Part model, mm, in its own coordinate system. Give positions to 0.01 mm unless a question says otherwise; leave off trailing zeros. Order: outer loops, then holes, each group sorted by start corner. A loop starts at its lowest first (then second) coordinate and runs counter-clockwise, first axis right, second up. Notation, with made-up numbers: (76.5, 14) - (93.5, 14) arc R15 ccw to (93.5, 20) - close; hole circle Ø2 at (39.5, 57.5). An arc over 180 degrees is marked (long way). Use a Markdown table: item, result. Add a question column.
from build123d import *

# Parameters (mm, degrees)
SKETCH_1_W         = 180
SKETCH_1_H         = 60
EXTRUDE_1_DEPTH    = 60
HOLE_WIZARD_M4_1_D = 4.8


with BuildPart() as part:
    # 草图1 → 凸台-拉伸1 (new body)
    with BuildSketch(Plane(origin=(0, 0, 0), x_dir=(1, 0, 0), z_dir=(0, 1, 0))):
        Rectangle(SKETCH_1_W, SKETCH_1_H)
    extrude(amount=EXTRUDE_1_DEPTH)

    # M4 间隙孔1 (through all)
    with Locations(Plane(origin=(0, 0, -30), x_dir=(-1, 0, 0), z_dir=(0, 0, -1))):
        with Locations((0, 30), (50, 30), (-50, 30)):
            Hole(HOLE_WIZARD_M4_1_D / 2)


solid = part.part
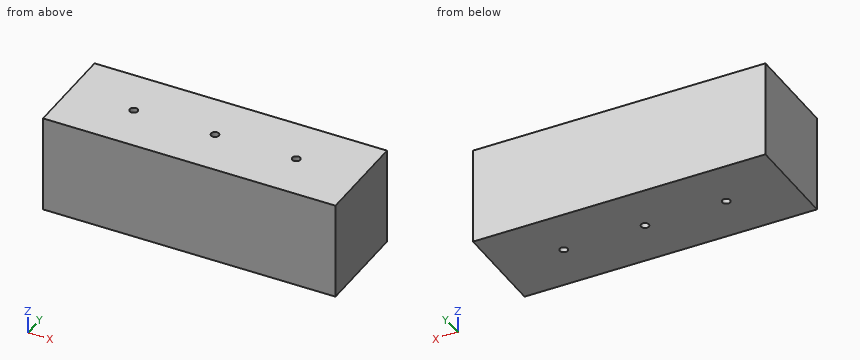
1. Cut at B-B (x = -50). Write the cut outline in (y, z), plus the area to 3 significant figures.
2. Pin check, flat tip, straight feed: P1, Ø3, axis at x = -50, y = 30, coming from the -Z side. Stop position of the tip, or through.
3. Drill centre lines: probe 1 along Y at (x, z) = (0, 6); probe 2 along X at (y, z) = (29, 27); probe 3 along X at (y, z) = (30.5, -25). Where is each one in solid material? Low to high. Write a range as [from, to].
4. Cut at A-A (y = 30). Write the cut outline in (x, z).
Responses:
| question | item | result |
|---|---|---|
| 1 | outline | (0, -30) - (27.6, -30) - (27.6, 30) - (0, 30) - close; (32.4, -30) - (60, -30) - (60, 30) - (32.4, 30) - close |
| 1 | area | 3,310 mm² |
| 2 | P1 | passes through |
| 3 | probe 1 | y = [0, 27.6], [32.4, 60] |
| 3 | probe 2 | x = [-90, -52.18], [-47.82, -2.18], [2.18, 47.82], [52.18, 90] |
| 3 | probe 3 | x = [-90, -52.35], [-47.65, -2.35], [2.35, 47.65], [52.35, 90] |
| 4 | outline | (-90, -30) - (-52.4, -30) - (-52.4, 30) - (-90, 30) - close; (-47.6, -30) - (-2.4, -30) - (-2.4, 30) - (-47.6, 30) - close; (2.4, -30) - (47.6, -30) - (47.6, 30) - (2.4, 30) - close; (52.4, -30) - (90, -30) - (90, 30) - (52.4, 30) - close |
